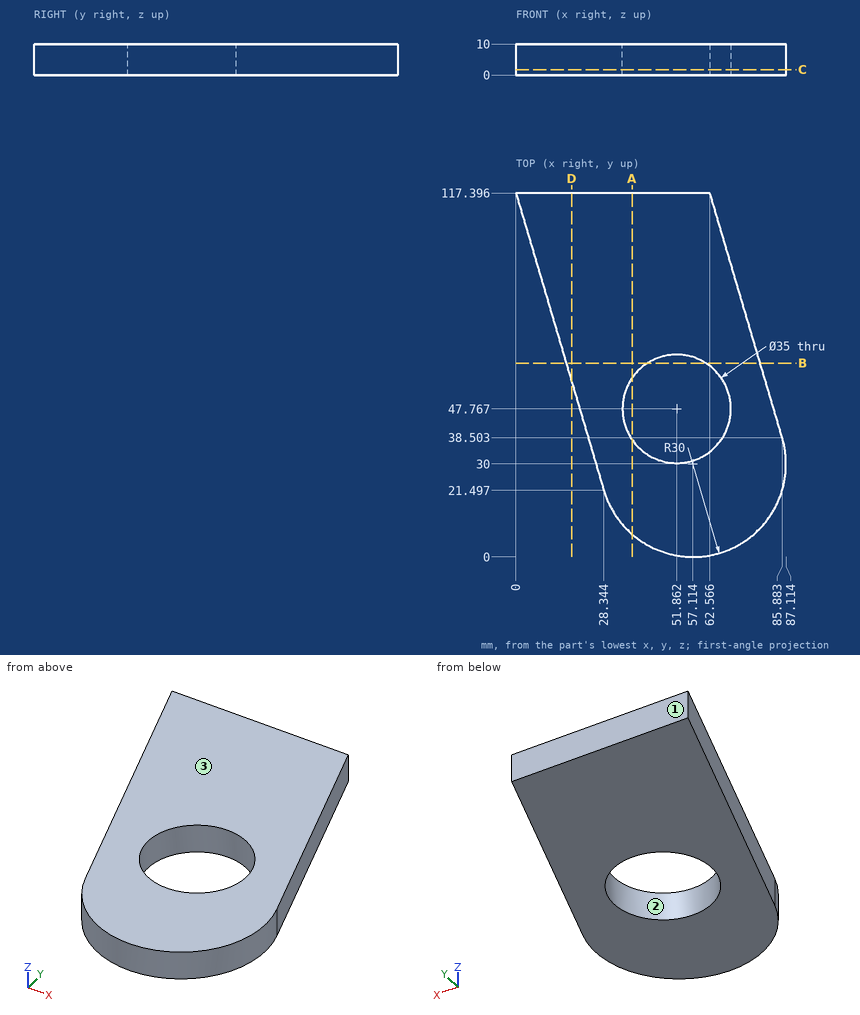
Verification items for this drawing (mm, ordinates from the low corner). Give positions to 0.01 mm unless a question says otherwise; leave off trailing zeros. Write each loop counter-clockwise with the first axis right and the second up, starting at its lowest first coordinate (ties: lowest second). Pieces come first, ordered by that corner, then holes.
1) Thickness scan on line 1 (X direction, y = 58, z = 5.5) (1 decimal); line 2 (Y direction, x = 56, z = 1.75) (1 decimal); line 3 (X direction, y = 57.5, z = 6.25) (1 decimal). Record the ranges inside material, lowest first.
Values follow:
line 1: x = 17.6 to 37.7, 66.1 to 80.1
line 2: y = 0 to 30.8, 64.8 to 117.4
line 3: x = 17.7 to 37.3, 66.4 to 80.3
2) Release check for a two-part mould opening along Y. For the marked faces 1, 2 and 3 record: released by +Y, released by -Y, zero draft, split by the parting line, or undercut.
Values follow:
face 1: released by +Y
face 2: undercut
face 3: zero draft
3) Go/stop test with flat-tipped pins: pin 1 Ø5 at (y, z) = (46.5, 5.5) entering from +X; pin 2 Ø6 at (y, z) = (70.5, 6) entering from -X; pin 3 Ø1 at (y, z) = (31, 8) entering from -X. Record where each tip stops, or that it passes through.
Values follow:
pin 1: stops at x = 84.26
pin 2: stops at x = 12.97
pin 3: stops at x = 25.39
4) Cross-section at D-D (x = 18). Record the boundary of the cut face in (y, z) (1 decimal).
Values follow:
outline: (56.5, 0) - (117.4, 0) - (117.4, 10) - (56.5, 10) - close
5) Cross-section at C-C (z = 1.75). Record the boundary of the cut face in (x, y) (1 decimal).
Values follow:
outline: (0, 117.4) - (28.3, 21.5) arc R30 ccw to (85.9, 38.5) - (62.6, 117.4) - close; hole circle Ø35 at (51.9, 47.8)
6) Cross-section at B-B (y = 62.5). Record the boundary of the cut face in (x, z) (1 decimal).
Values follow:
outline: (16.2, 0) - (42.4, 0) - (42.4, 10) - (16.2, 10) - close; (61.3, 0) - (78.8, 0) - (78.8, 10) - (61.3, 10) - close
7) Cross-section at A-A (x = 37.5). Record the boundary of the cut face in (y, z) (1 decimal).
Values follow:
outline: (7.3, 0) - (37.8, 0) - (37.8, 10) - (7.3, 10) - close; (57.8, 0) - (117.4, 0) - (117.4, 10) - (57.8, 10) - close
